Input: part model. Units: mm. Frame: model coordinates. Coordinates: 2 decimals unless noted, no trailing zeros. Write item = value, one per line. Start each with the question number.
from build123d import *

# Parameters (mm, degrees)
SKETCH1_W               = 10.85
SKETCH1_H               = 10.85
BOSS_EXTRUDE1_DEPTH     = 1000
MIRROR2_COPY_1_SKETCH_W = 10.85
MIRROR2_COPY_1_SKETCH_H = 10.85
MIRROR2_COPY_1_DEPTH    = 1000


with BuildPart() as part:
    # Sketch1 → Boss-Extrude1 (new body)
    with BuildSketch(Plane(origin=(0, 0, 0), x_dir=(1, 0, 0), z_dir=(0, 1, 0))):
        with BuildLine():
            Line((-4.3, 20), (-19.5, 20))
            ThreePointArc((-19.5, 20), (-19.853553391, 19.853553391), (-20, 19.5))
            Line((-20, 19.5), (-20, 4.3))
            Line((-20, 4.3), (-19.05, 4.3))
            Line((-19.05, 4.3), (-19.05, 7.25))
            Line((-19.05, 7.25), (-7.921751442, 7.25))
            Line((-7.921751442, 7.25), (-6.2, 5.528248558))
            Line((-6.2, 5.528248558), (-6.2, 0))
            Line((-6.2, 0), (-5.3, 0))
            ThreePointArc((-5.3, 0), (-5.066731596, 1.555066215), (-4.387460025, 2.973246463))
            Line((-4.387460025, 2.973246463), (-5.091168825, 3.676955262))
            ThreePointArc((-5.091168825, 3.676955262), (-5.091168825, 5.091168825), (-3.676955262, 5.091168825))
            Line((-3.676955262, 5.091168825), (-2.973246463, 4.387460025))
            ThreePointArc((-2.973246463, 4.387460025), (-1.555066215, 5.066731596), (0, 5.3))
            Line((0, 5.3), (0, 6.2))
            Line((0, 6.2), (-5.528248558, 6.2))
            Line((-5.528248558, 6.2), (-7.25, 7.921751442))
            Line((-7.25, 7.921751442), (-7.25, 19.05))
            Line((-7.25, 19.05), (-4.3, 19.05))
            Line((-4.3, 19.05), (-4.3, 20))
        make_face()
        with Locations((-13.625, 13.625)):
            Rectangle(SKETCH1_W, SKETCH1_H, mode=Mode.SUBTRACT)
    boss_extrude1 = extrude(amount=BOSS_EXTRUDE1_DEPTH)

    # Mirror1: Boss-Extrude1 across plane
    add(boss_extrude1.mirror(Plane(origin=(0, 0, 0), x_dir=(0, 0, 1), z_dir=(1, 0, 0))))

    # Mirror2: Boss-Extrude1 across plane
    add(boss_extrude1.mirror(Plane.XY))

    # Mirror2 copy 1 sketch → Mirror2 copy 1 (add)
    with BuildSketch(Plane(origin=(0, 0, 0), x_dir=(-1, 0, 0), z_dir=(0, 1, 0))):
        with BuildLine():
            Line((-4.3, 20), (-19.5, 20))
            ThreePointArc((-19.5, 20), (-19.853553391, 19.853553391), (-20, 19.5))
            Line((-20, 19.5), (-20, 4.3))
            Line((-20, 4.3), (-19.05, 4.3))
            Line((-19.05, 4.3), (-19.05, 7.25))
            Line((-19.05, 7.25), (-7.921751442, 7.25))
            Line((-7.921751442, 7.25), (-6.2, 5.528248558))
            Line((-6.2, 5.528248558), (-6.2, 0))
            Line((-6.2, 0), (-5.3, 0))
            ThreePointArc((-5.3, 0), (-5.066731596, 1.555066215), (-4.387460025, 2.973246463))
            Line((-4.387460025, 2.973246463), (-5.091168825, 3.676955262))
            ThreePointArc((-5.091168825, 3.676955262), (-5.091168825, 5.091168825), (-3.676955262, 5.091168825))
            Line((-3.676955262, 5.091168825), (-2.973246463, 4.387460025))
            ThreePointArc((-2.973246463, 4.387460025), (-1.555066215, 5.066731596), (0, 5.3))
            Line((0, 5.3), (0, 6.2))
            Line((0, 6.2), (-5.528248558, 6.2))
            Line((-5.528248558, 6.2), (-7.25, 7.921751442))
            Line((-7.25, 7.921751442), (-7.25, 19.05))
            Line((-7.25, 19.05), (-4.3, 19.05))
            Line((-4.3, 19.05), (-4.3, 20))
        make_face()
        with Locations((-13.625, 13.625)):
            Rectangle(MIRROR2_COPY_1_SKETCH_W, MIRROR2_COPY_1_SKETCH_H, mode=Mode.SUBTRACT)
    extrude(amount=MIRROR2_COPY_1_DEPTH)


solid = part.part
Item 1: Ray query, line 1 (Z direction, x = -5.5, y = 630); line 2 (X direction, y = 400.5, z = -14.5). Return the intervals inside material, ascending.
Item 2: Pin query (flat end, axial travel): pin 1 (10 mm diameter, centred on x = 12, z = -0.5, fed in from +Y). Return the tip coordinate at first contact, or that it passes through.
Item 3: Cut plane A-A on y = 774. State how many separate pieces and enclosed holes the cut face has, plus the area to 3 significant figures.
Recorded:
q1.line_1 = -20 to -19.05, -6.2 to 6.2, 19.05 to 20
q1.line_2 = -20 to -19.05, -8.2 to -7.25, 7.25 to 8.2, 19.05 to 20
q2.pin_1 = through
q3.separate_pieces = 1
q3.enclosed_holes = 5
q3.area = 261 mm²
